from build123d import *

# Parameters (mm, degrees)
BOSS_EXTRUDE1_DEPTH      = 30
SKETCH4_W                = 15
SKETCH4_H                = 340
CUT_EXTRUDE1_DEPTH       = 415.3971525
M16_TAPPED_HOLE3_D       = 14
M16_TAPPED_HOLE3_DEPTH   = 60
M16_TAPPED_HOLE3_TIP     = 4.206024333
M16_TAPPED_HOLE2_D       = 14
M16_TAPPED_HOLE2_DEPTH   = 50
M16_TAPPED_HOLE2_TIP     = 4.206024333
M8_TAPPED_HOLE1_D        = 6.8
F_9_0_9_DIAMETER_HOLE1_D = 9


with BuildPart() as part:
    # Sketch1 → Boss-Extrude1 (new body)
    with BuildSketch(Plane.XY):
        with BuildLine():
            Line((0, 0), (235, 0))
            Line((235, 0), (235, 20))
            ThreePointArc((235, 20), (234.444340269, 26.644096684), (232.792798963, 33.103600519))
            Line((232.792798963, 33.103600519), (207.207201037, 106.896399481))
            ThreePointArc((207.207201037, 106.896399481), (205.555659731, 113.355903316), (205, 120))
            Line((205, 120), (205, 220))
            ThreePointArc((205, 220), (205.555659731, 226.644096684), (207.207201037, 233.103600519))
            Line((207.207201037, 233.103600519), (232.792798963, 306.896399481))
            ThreePointArc((232.792798963, 306.896399481), (234.444340269, 313.355903316), (235, 320))
            Line((235, 320), (235, 340))
            Line((235, 340), (0, 340))
            Line((0, 340), (0, 320))
            ThreePointArc((0, 320), (0.555659731, 313.355903316), (2.207201037, 306.896399481))
            Line((2.207201037, 306.896399481), (27.792798963, 233.103600519))
            ThreePointArc((27.792798963, 233.103600519), (29.444340269, 226.644096684), (30, 220))
            Line((30, 220), (30, 120))
            ThreePointArc((30, 120), (29.444340269, 113.355903316), (27.792798963, 106.896399481))
            Line((27.792798963, 106.896399481), (2.207201037, 33.103600519))
            ThreePointArc((2.207201037, 33.103600519), (0.555659731, 26.644096684), (0, 20))
            Line((0, 20), (0, 0))
        make_face()
        with BuildLine():
            Line((92.5, 85), (92.5, 245))
            ThreePointArc((92.5, 245), (117.5, 270), (142.5, 245))
            Line((142.5, 245), (142.5, 85))
            ThreePointArc((142.5, 85), (117.5, 60), (92.5, 85))
        make_face(mode=Mode.SUBTRACT)
    extrude(amount=BOSS_EXTRUDE1_DEPTH)

    # Sketch4 → Cut-Extrude1 (cut, through all)
    with BuildSketch(Plane.XY.offset(30)):
        with Locations((7.5, 170)):
            Rectangle(SKETCH4_W, SKETCH4_H)
    extrude(amount=-CUT_EXTRUDE1_DEPTH, mode=Mode.SUBTRACT)

    # M16 Tapped Hole3
    with Locations(Plane(origin=(0, 0, 0), x_dir=(-1, 0, 0), z_dir=(0, -1, 0))):
        with Locations((-215, -15), (-65, -15), (-140, -15)):
            Hole(M16_TAPPED_HOLE3_D / 2, depth=M16_TAPPED_HOLE3_DEPTH)
            with Locations((0, 0, -(M16_TAPPED_HOLE3_DEPTH + M16_TAPPED_HOLE3_TIP / 2))):  # 118° drill point
                Cone(0, M16_TAPPED_HOLE3_D / 2, M16_TAPPED_HOLE3_TIP, mode=Mode.SUBTRACT)

    # M16 Tapped Hole2
    with Locations(Plane(origin=(0, 340, 0), x_dir=(1, 0, 0), z_dir=(0, 1, 0))):
        with Locations((215, -15), (65, -15), (127, -15)):
            Hole(M16_TAPPED_HOLE2_D / 2, depth=M16_TAPPED_HOLE2_DEPTH)
            with Locations((0, 0, -(M16_TAPPED_HOLE2_DEPTH + M16_TAPPED_HOLE2_TIP / 2))):  # 118° drill point
                Cone(0, M16_TAPPED_HOLE2_D / 2, M16_TAPPED_HOLE2_TIP, mode=Mode.SUBTRACT)

    # M8 Tapped Hole1 (through all)
    with Locations(Plane.XY.offset(30)):
        with Locations((25.5, 324), (49.5, 324), (189.5, 324), (165.5, 324)):
            Hole(M8_TAPPED_HOLE1_D / 2)

    # Ø9.0 (9) Diameter Hole1 (through all)
    with Locations(Plane.XY.offset(30)):
        with Locations((197.5, 15), (197.5, 35), (32.5, 15), (32.5, 35)):
            Hole(F_9_0_9_DIAMETER_HOLE1_D / 2)


solid = part.part
CAD build for the part. Positions are in the model's coordinates, mm. A direction names the side the tool comes from. Coordinates: 2 decimals unless noted, no trailing zeros. Order: outer loops, then holes, each group sorted by start corner. A loop starts at its lowest first (then second) coordinate and runs counter-clockwise, first axis right, second up. Notation, with made-up numbers: (31.5, 49.5) -> (73.5, 49.5) arc R18 ccw to (73.5, 77.5) -> close; hole circle Ø2 at (78.5, -33). An arc over 180 degrees is marked (long way). Answer in a Markdown table with one row per item.
1) Drill centre lines: line 1 (Y direction, x = 197.5, z = 8.25); line 2 (Z direction, x = 65, y = 25); line 3 (X direction, y = 33.5, z = 10). Where is each one in solid material? Low to high.
Check values:
| item | result |
|---|---|
| line 1 | 0 to 10.5, 19.5 to 30.5, 39.5 to 340 |
| line 2 | 0 to 8, 22 to 30 |
| line 3 | 15 to 28.26, 36.74 to 60.1, 69.9 to 135.1, 144.9 to 193.26, 201.74 to 210.1, 219.9 to 232.66 |
2) Band-saw the part on C-C (y = 171.5). List the corners of the cut face in (x, z).
Check values:
| item | result |
|---|---|
| outline | (30, 0) -> (92.5, 0) -> (92.5, 30) -> (30, 30) -> close; (142.5, 0) -> (205, 0) -> (205, 30) -> (142.5, 30) -> close |
3) Band-saw the part on B-B (x = 189.5). List the corners of the cut face in (y, z).
Check values:
| item | result |
|---|---|
| outline | (0, 0) -> (320.6, 0) -> (320.6, 30) -> (0, 30) -> close; (327.4, 0) -> (340, 0) -> (340, 30) -> (327.4, 30) -> close |
4) Flat gauge pins, fed straight in: P1, Ø10.5, axis at x = 32.5, y = 35, coming from the -Z side; P2, Ø11, axis at x = 140, z = 15, coming from the -Y side; P3, Ø9, axis at y = 177, z = 9.5, coming from the +X side; P4, Ø4, axis at y = 136, z = 7.5, coming from the -X side. Where does each tip first touch, or does it go through?
Check values:
| item | result |
|---|---|
| P1 | z = 0 |
| P2 | y = 60.9 |
| P3 | x = 205 |
| P4 | x = 30 |
5) Mould opens along Y. For faces 6 (the face through (220.18, 69.48, 14.79)), 7 (the face through (30, 171, 15)), 8 (the face through (15, 305, 15)), 9 (the face through (123, 0, 15)) say: pulls with the +Y half, pulls with the -Y half, needs draft (parallel to the pull), parting line crosses it, or undercut.
Check values:
| item | result |
|---|---|
| face 6 | undercut |
| face 7 | undercut |
| face 8 | needs draft |
| face 9 | pulls with the -Y half |
6) Which spindle directions (+Z, -Z, +X, -X, +Y, -Y) get a long thin tool onto all of the face, cutting with end or side? Do faces 1 (the face through (118.05, 60.006, 14.79)), 2 (the face through (58.534, 314.65, 17.681)), 3 (the face through (134.445, 30.42, 19.259)), 4 (the face through (205.57, 113.26, 14.79)), 5 (the face through (21.307, 251.81, 14.79)). Say none if no direction does.
Check values:
| item | result |
|---|---|
| face 1 | +Z, -Z |
| face 2 | +Y |
| face 3 | -Y |
| face 4 | +Z, -Z, +X |
| face 5 | +Z, -Z, -X |
7) Band-saw the part on A-A (y = 324). List the corners of the cut face in (x, z), and give its area (3 significant figures).
Check values:
| item | result |
|---|---|
| outline | (15, 0) -> (22.1, 0) -> (22.1, 30) -> (15, 30) -> close; (28.9, 0) -> (46.1, 0) -> (46.1, 30) -> (28.9, 30) -> close; (52.9, 0) -> (162.1, 0) -> (162.1, 30) -> (52.9, 30) -> close; (168.9, 0) -> (186.1, 0) -> (186.1, 30) -> (168.9, 30) -> close; (192.9, 0) -> (235, 0) -> (235, 30) -> (192.9, 30) -> close; hole circle Ø14 at (65, 15); hole circle Ø14 at (127, 15); hole circle Ø14 at (215, 15) |
| area | 5,320 mm2 |
